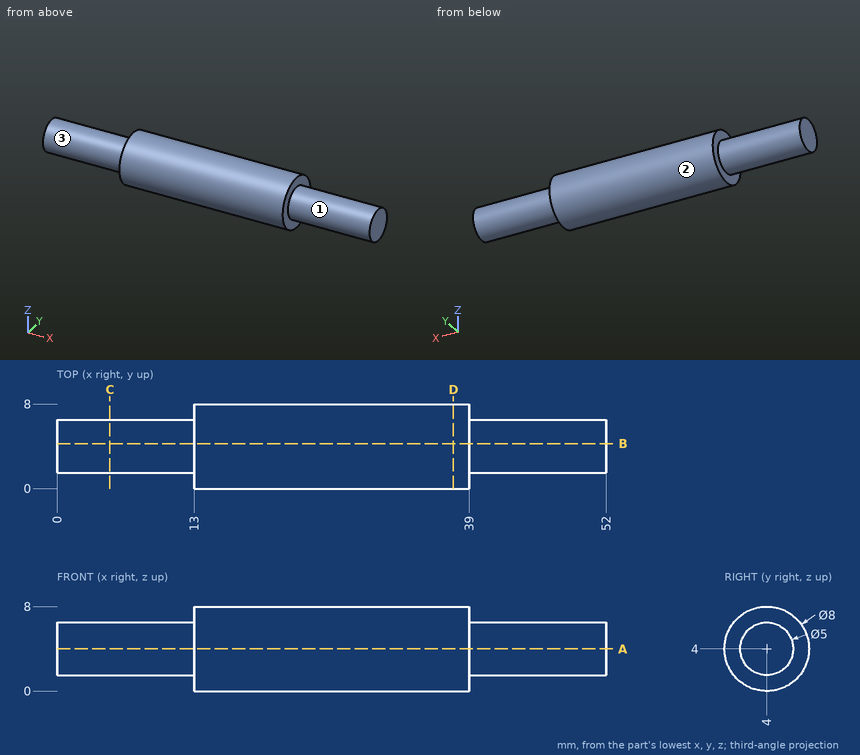
Design review of the part shown in the three views and the two pictorial views. Dimensions are in mm from the part's minimum x, y and z. A direction names the side the tool comes from. Give positions to 0.01 mm unless a question says otherwise; leave off trailing zeros. Write each loop counter-clockwise with the first axis right and the second up, starting at its lowest first coordinate (ties: lowest second). Pieces come first, ordered by that corner, then holes. Notation, with made-up numbers: M 43,62 L 73,62 A22 ccw 73,86 Z; hole C 42.25,49 d9. An arc over 180 degrees is marked long. Return JSON: item names as keys, results as strings. Group by question number.
Item 1: Wall thickness on line 1 along X through (y, z) = (6, 6); line 2 along Z through (x, y) = (31.5, 4.25); line 3 along Y through (x, z) = (41, 4): over which ranges is each line inside the solid? List them lowest first.
Item 2: Clearance check with flat-ended pins moving along their axes: pin 1 Ø1 at (x, z) = (19, 1.5) entering from -Y; pin 2 Ø2 at (x, z) = (23.5, 7) entering from +Y. State where each tip first meets the part, or that it passes through.
Item 3: Take a section at A-A (z = 4). Give the boundary of the cut face in (x, y), plus the area to 3 significant figures.
Item 4: Take a section at B-B (y = 4.25). Give the boundary of the cut face in (x, z), plus the area to 3 significant figures.
Item 5: Tool access review of the marked faces 1, 2 and 3: name each direction out of +Z, -Z, +X, -X, +Y, -Y from which nothing blocks a thin tool from reaching the whole face with its end or side.
Item 6: Take a section at C-C (x = 5). Give the boundary of the cut face in (y, z), plus the area to 3 significant figures.
Item 7: Take a section at D-D (x = 37.5). Give the boundary of the cut face in (y, z), plus the area to 3 significant figures.
Return value:
{
 "1": {"line 1": "x = 13 to 39", "line 2": "z = 0.01 to 7.99", "line 3": "y = 1.5 to 6.5"},
 "2": {"pin 1": "stops at y = 0.54", "pin 2": "stops at y = 7.46"},
 "3": {"outline": "M 0,1.5 L 13,1.5 L 13,0 L 39,0 L 39,1.5 L 52,1.5 L 52,6.5 L 39,6.5 L 39,8 L 13,8 L 13,6.5 L 0,6.5 Z", "area": "338 mm2"},
 "4": {"outline": "M 0,1.51 L 13,1.51 L 13,0.01 L 39,0.01 L 39,1.51 L 52,1.51 L 52,6.49 L 39,6.49 L 39,7.99 L 13,7.99 L 13,6.49 L 0,6.49 Z", "area": "337 mm2"},
 "5": {"face 1": "+X", "face 2": "+X, -X", "face 3": "-X"},
 "6": {"outline": "C 4,4 d5", "area": "19.6 mm2"},
 "7": {"outline": "C 4,4 d8", "area": "50.3 mm2"}
}
